from build123d import *

# Parameters (mm, degrees)
SKETCH1_W           = 1270
SKETCH1_H           = 240
BOSS_EXTRUDE1_DEPTH = 20
SKETCH3_W           = 64
SKETCH3_H           = 30
BOSS_EXTRUDE2_DEPTH = 240


with BuildPart() as part:
    # Sketch1 → Boss-Extrude1 (new body)
    with BuildSketch(Plane.XY):
        with Locations((635, 120)):
            Rectangle(SKETCH1_W, SKETCH1_H)
    extrude(amount=BOSS_EXTRUDE1_DEPTH)

    # Sketch3 → Boss-Extrude2 (add)
    with BuildSketch(Plane.XZ):
        with Locations((32, 10)):
            Rectangle(SKETCH3_W, SKETCH3_H)
        with Locations((336, 10)):
            Rectangle(SKETCH3_W, SKETCH3_H)
        with Locations((640, 10)):
            Rectangle(SKETCH3_W, SKETCH3_H)
        with Locations((944, 10)):
            Rectangle(SKETCH3_W, SKETCH3_H)
        with Locations((1248, 10)):
            Rectangle(SKETCH3_W, SKETCH3_H)
    extrude(amount=-BOSS_EXTRUDE2_DEPTH)


solid = part.part
Here's how the part is built. I have some questions about the finished solid (model axes, mm). A direction names the side the tool comes from. Give positions to 0.01 mm unless a question says otherwise; leave off trailing zeros. Order: outer loops, then holes, each group sorted by start corner. A loop starts at its lowest first (then second) coordinate and runs counter-clockwise, first axis right, second up. Notation, with made-up numbers: (27, 53.5) -> (77, 53.5) arc R26 cw to (77, 69.5) -> close; hole circle Ø10 at (59.25, 62). An arc over 180 degrees is marked (long way). Use a Markdown table: item, result. Add a question column.
Item 1: For faces 5 (the face through (944, 118, -5)), 6 (the face through (1094, 122, 20)), 7 (the face through (182, 122, 0)), which set-ups out of +Z, -Z, +X, -X, +Y, -Y let a thin tool reach every point of the face, with its end or its side?
Item 2: I need wall thicknesses on line 1 (X direction, y = 202, z = 24); line 2 (Z direction, x = 1057.5, y = 142). Which ranges of each line are inside material? Lowest first, please.
Item 3: Imagine slicing it at A-A on x = 418.5. Please give me the cut outline in (y, z), plus the area to 3 significant figures.
Item 4: Will these pins go through, and if not, where does the flat tip stop? pin 1 (1.5 mm diameter, centred on x = 175, y = 77.5, fed in from +Z); pin 2 (6 mm diameter, centred on x = 1065.5, y = 169, fed in from -Z).
Item 5: If we mould it in two halves opening along X, with no side actions, what happens to faces 1 (the face through (486, 122, 0)), 2 (the face through (32, 118, -5)), 3 (the face through (0, 118, 10)), 4 (the face through (182, 122, 20))? For each: pulls with the +X half, pulls with the -X half, needs draft (parallel to the pull), parting line crosses it, or undercut.
Data:
| question | item | result |
|---|---|---|
| 1 | face 5 | -Z, +X, -X, +Y, -Y |
| 1 | face 6 | +Z, +Y, -Y |
| 1 | face 7 | -Z, +Y, -Y |
| 2 | line 1 | x = 0 to 64, 304 to 368, 608 to 672, 912 to 976, 1216 to 1280 |
| 2 | line 2 | z = 0 to 20 |
| 3 | outline | (0, 0) -> (240, 0) -> (240, 20) -> (0, 20) -> close |
| 3 | area | 4,800 mm² |
| 4 | pin 1 | stops at z = 20 |
| 4 | pin 2 | stops at z = 0 |
| 5 | face 1 | undercut |
| 5 | face 2 | needs draft |
| 5 | face 3 | pulls with the -X half |
| 5 | face 4 | undercut |
